from build123d import *

# Parameters (mm, degrees)
BOSS_EXTRUDE1_START = -3.5
SKETCH4_R           = 1
BOSS_EXTRUDE1_DEPTH = 3.5
SKETCH5_R           = 5.237604307
SKETCH5_R_2         = 4
CUT_EXTRUDE1_DEPTH  = 1
CUT_EXTRUDE1_DRAFT  = -55
CHAMFER1_SIZE       = 0.5


with BuildPart() as part:
    # Sketch3 → Revolve1 (revolve)
    with BuildSketch(Plane(origin=(0, 0, 0), x_dir=(0, 0, -1), z_dir=(1, 0, 0)), mode=Mode.PRIVATE) as revolve1_sk:
        Polygon((0, 2.5), (-3.5, 2.5), (-3.5, 1), (25, 1), (25, 2.5), align=None)
    revolve(revolve1_sk.sketch.rotate(Axis((0, 0, 3.5), (0, 0, -1)), 180), axis=Axis((0, 0, 3.5), (0, 0, -1)))

    # Sketch4 → Boss-Extrude1 (add)
    with BuildSketch(Plane.XY.offset(3.5).offset(BOSS_EXTRUDE1_START)):
        Polygon((2.309401077, 4), (-2.309401077, 4), (-4.618802154, 0), (-2.309401077, -4), (2.309401077, -4), (4.618802154, 0), align=None)
        with Locations(Location((0, 0, 0), (0, 0, 270))):
            Circle(SKETCH4_R, mode=Mode.SUBTRACT)
    extrude(amount=BOSS_EXTRUDE1_DEPTH)


with BuildPart() as cut_extrude1_tool:
    # Sketch5 → Cut-Extrude1 (with draft: the straight prism first)
    with BuildSketch(Plane.XY.offset(3.5)):
        Circle(SKETCH5_R)
        Circle(SKETCH5_R_2, mode=Mode.SUBTRACT)
    extrude(amount=-CUT_EXTRUDE1_DEPTH)
    # Cut-Extrude1: the draft: its side faces are tilted about the plane it starts from
    cut_extrude1_sides = [cut_extrude1_tool.faces().sort_by_distance(p)[0] for p in [
        (-5.237604307, 0, 3),
        (-4, 0, 3),
    ]]
    draft(cut_extrude1_sides, Plane.XY.offset(3.5), CUT_EXTRUDE1_DRAFT)


with BuildPart() as part_1:
    add(part.part)

    # Cut-Extrude1: cut by cut_extrude1_tool
    add(cut_extrude1_tool.part, mode=Mode.SUBTRACT)

    # Chamfer1
    chamfer1_edges = [part_1.edges().sort_by_distance(p)[0] for p in [
        (0, 2.5, -25),
    ]]
    chamfer(chamfer1_edges, length=CHAMFER1_SIZE)


solid = part_1.part
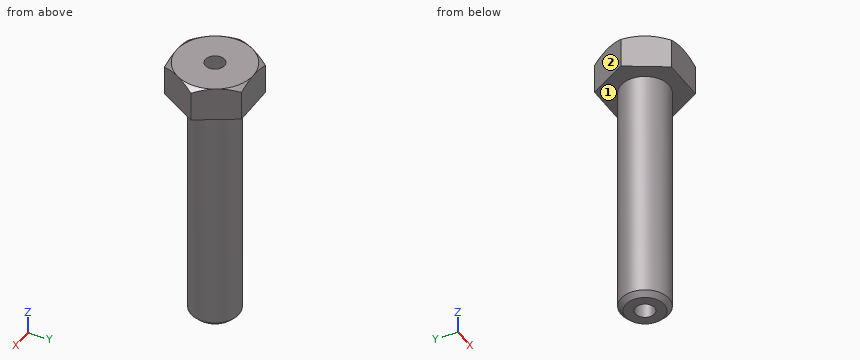
For this review, take the finished solid that the model builds, in its own axes (mm). Face numbers are marked on the shaded views. A direction names the side the tool comes from. Round coordinates to 2 decimals unless told otherwise and drop trailing zeros. Loops run counter-clockwise (first coordinate to the right, second up) from the corner with the lowest first, then second, coordinate; pieces in that order, holes last. Notation, with made-up numbers: (23, 23) - (36, 23) arc R24 ccw to (36, 59) - close; hole circle Ø10 at (78.25, 60.5). An arc over 180 degrees is marked (long way). One line per question, with ' | ' between items.
Q1. For pin 1 (2 mm diameter, centred on y = 3, z = -13.5, fed in from -X); pin 2 (4 mm diameter, centred on y = 2, z = -9.5, fed in from -X); pin 3 (1.5 mm diameter, centred on y = -2.5, z = -17, fed in from +X), all flat-tipped, find the tip position at first contact; note any pin that passes through.
Taken from the geometry:
pin 1: stops at x = -1.5 | pin 2: stops at x = -2.5 | pin 3: stops at x = 1.79
Q2. Take a section at A-A (z = 0.5). Give the boundary of the cut face in (x, y).
Taken from the geometry:
outline: (-4.62, 0) - (-2.31, -4) - (2.31, -4) - (4.62, 0) - (2.31, 4) - (-2.31, 4) - close; hole circle Ø2 at (0, 0)
Q3. Tool access review of the marked faces 1 and 2: name each direction out of +Z, -Z, +X, -X, +Y, -Y from which nothing blocks a thin tool from reaching the whole face with its end or side.
Taken from the geometry:
face 1: -Z | face 2: +Z, -Z, -X, +Y
Q4. For line 1 along X through (y, z) = (0, -10); line 2 along Y through (x, z) = (-1.5, -23.5), list the stretches that pass through material, from the lowest coordinate up. Write a range as [from, to].
Taken from the geometry:
line 1: x = [-2.5, -1], [1, 2.5] | line 2: y = [-2, 2]
Q5. Take a section at B-B (z = -10). Give the boundary of the cut face in (x, y), and give its area (3 significant figures).
Taken from the geometry:
outline: circle Ø5 at (0, 0); hole circle Ø2 at (0, 0) | area: 16.5 mm²
